Build history of the part. All positions in model axes, mm. Coordinates: 2 decimals unless noted, no trailing zeros. Order: outer loops, then holes, each group sorted by start corner. A loop starts at its lowest first (then second) coordinate and runs counter-clockwise, first axis right, second up. Notation, with made-up numbers: (39, -35) - (75, -35) arc R16 ccw to (75, -16) - close; hole circle Ø7 at (12, -8.75). An arc over 180 degrees is marked (long way). One line per item, written item: value.
from build123d import *

# Parameters (mm, degrees)
BOSS_EXTRUDE1_DEPTH = 30


with BuildPart() as part:
    # Sketch1 → Boss-Extrude1 (new body)
    with BuildSketch(Plane.XY):
        Polygon((0, 0), (0, 72.5), (5, 77.5), (75, 77.5), (80, 72.5), (80, 67.5), (20, 0), align=None)
    extrude(amount=BOSS_EXTRUDE1_DEPTH)


solid = part.part
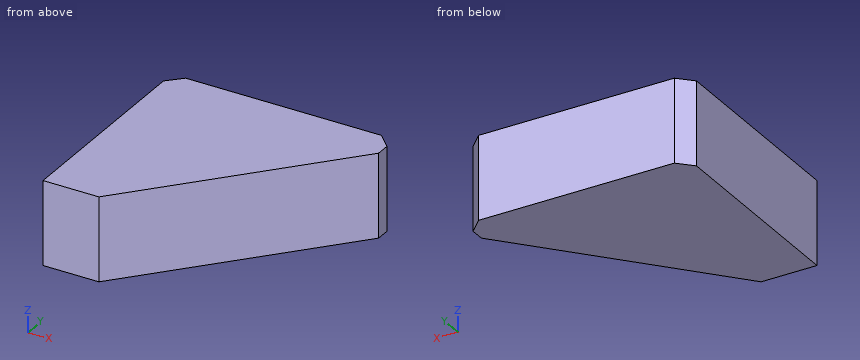
1. Band-saw the part on A-A, the plane z = 13.5. Give the cut face in (x, y).
Values found:
outline: (0, 0) - (20, 0) - (80, 67.5) - (80, 72.5) - (75, 77.5) - (5, 77.5) - (0, 72.5) - close
2. Band-saw the part on C-C, the plane y = 27.5. Give the cut face in (x, z).
Values found:
outline: (0, 0) - (44.44, 0) - (44.44, 30) - (0, 30) - close
3. Band-saw the part on B-B, the plane x = 68. Give the cut face in (y, z), and give its area (3 significant figures).
Values found:
outline: (54, 0) - (77.5, 0) - (77.5, 30) - (54, 30) - close
area: 705 mm2
4. Probe line 1 along X through (y, z) = (46, 3.25); line 2 along Y through (x, z) = (55, 19) (3 decimals); line 3 along X through (y, z) = (14, 26). List the from-to ranges inside material, lowest first.
Values found:
line 1: x = 0 to 60.89
line 2: y = 39.375 to 77.5
line 3: x = 0 to 32.44
5. Flat gauge pins, fed straight in: P1, Ø4, axis at y = 66.5, z = 20, coming from the -X side; P2, Ø12, axis at x = 39, z = 12, coming from the -Y side (3 decimals); P3, Ø10, axis at y = 10, z = 20, coming from the +X side; P4, Ø4, axis at y = 18, z = 7.5, coming from the +X side. Where does each tip first touch, or does it go through?
Values found:
P1: stops at x = 0
P2: stops at y = 14.625
P3: stops at x = 33.33
P4: stops at x = 37.78
